Could you check a few things on this model? Use its own coordinates, in mm. A direction names the side the tool comes from. Round coordinates to 2 decimals unless told otherwise and drop trailing zeros. Order: outer loops, then holes, each group sorted by start corner. A loop starts at its lowest first (then second) coordinate and runs counter-clockwise, first axis right, second up. Notation, with made-up numbers: M -30.75,1 L 26.25,1 A17 ccw 26.25,17 Z; hole C 88.25,44.25 d3. An arc over 180 degrees is marked long. Write each question's results on one line, items separated by ' | '. Start each with the question number.
1. Suppose I cut it at A-A on y = 0. Write out the boundary of the cut face in (x, z), and give its area (3 significant figures).
2. Suppose I cut it at B-B on z = 4.5. Write out the boundary of the cut face in (x, y), and give its area (3 significant figures).
3. For faces 1 (the flat face through (1, 22.5, 4)), 2 (the cylindrical face through (21.1, -1.5, 2)), 3 (the cylindrical face through (9.89, 0.33, -1.05)), which set-ups out of +Z, -Z, +X, -X, +Y, -Y let a thin tool reach every point of the face, with its end or its side?
4. I'm going to push flat-ended pins straight in: pin 1 (2 mm diameter, centred on x = 20, z = 0, fed in from +Y); pin 2 (2 mm diameter, centred on x = 2.5, y = 19.5, fed in from +Z); pin 3 (0.8 mm diameter, centred on y = 0, z = 3.5, fed in from -X); pin 4 (2 mm diameter, centred on x = 22, y = 0, fed in from +Z). Where does each tip first touch, or does it pass through?
5. We'd pull the mould along Y, two halves only. Please class faces 4 (the flat face through (12, -27.5, 0)), 5 (the conical face through (19.72, 16.58, -0.04)), 6 (the flat face through (4.5, -19, 4)): released by +Y, released by -Y, zero draft, split by the parting line, or undercut.
6. Please list where these lines run through material, in increasing order: L1, parallel to X at y = 21.5, z = 0; L2, parallel to Y at x = 2, z = 0.25; L3, parallel to Y at x = 13, z = 0.
from build123d import *

# Parameters (mm, degrees)
SKETCH_1_W                  = 12
SKETCH_1_H                  = 55
EXTRUDE_1_DEPTH             = 25
SKETCH_2_R                  = 1.1
CUT_EXTRUDE_1_DEPTH         = 25
SKETCH_3_R                  = 2.5
CUT_EXTRUDE_2_DEPTH         = 8
SKETCH_4_W                  = 24
SKETCH_4_H                  = 3
CUT_EXTRUDE_3_DEPTH         = 6
HOLE_WIZARD_M4_1_AT_2_COUNT = 2
HOLE_WIZARD_M4_1_AT_2_PITCH = 15
FILLET_1_R                  = 1
CUT_EXTRUDE_4_DEPTH         = 4
HOLE_WIZARD_M3_1_D          = 2.5
FILLET_2_R                  = 1


with BuildPart() as part:
    # 草图1 → 凸台-拉伸1 (new body)
    with BuildSketch(Plane(origin=(0, 0, 0), x_dir=(0, 0, -1), z_dir=(1, 0, 0))):
        Rectangle(SKETCH_1_W, SKETCH_1_H)
    extrude(amount=EXTRUDE_1_DEPTH)

    # 草图2 → 切除-拉伸1 (cut)
    with BuildSketch(Plane(origin=(25, 0, 0), x_dir=(0, 0, -1), z_dir=(1, 0, 0))):
        Circle(SKETCH_2_R)
    extrude(amount=-CUT_EXTRUDE_1_DEPTH, mode=Mode.SUBTRACT)

    # 草图3 → 切除-拉伸2 (cut)
    with BuildSketch(Plane(origin=(25, 0, 0), x_dir=(0, 0, -1), z_dir=(1, 0, 0))):
        Circle(SKETCH_3_R)
    extrude(amount=-CUT_EXTRUDE_2_DEPTH, mode=Mode.SUBTRACT)

    # 草图4 → 切除-拉伸3 (cut)
    with BuildSketch(Plane.XY.offset(6)):
        Rectangle(SKETCH_4_W, SKETCH_4_H)
    extrude(amount=-CUT_EXTRUDE_3_DEPTH, mode=Mode.SUBTRACT)

    # 草图7 → M4 螺纹孔1 (revolve, cut)
    with BuildSketch(Plane(origin=(5, 27.5, 0), x_dir=(0, 0, 1), z_dir=(1, 0, 0))):
        Polygon((0, 0), (0, 11.091420021), (1.65, 10.1), (1.65, 0), align=None)
    hole_wizard_m4_1 = revolve(axis=Axis((5, 33.85, 0), (0, -1, 0)), mode=Mode.SUBTRACT)

    # M4 螺纹孔1 at 2: M4 螺纹孔1 ×2
    with Locations(*[(i * HOLE_WIZARD_M4_1_AT_2_PITCH, 0, 0) for i in range(1, HOLE_WIZARD_M4_1_AT_2_COUNT)]):
        add(hole_wizard_m4_1, mode=Mode.SUBTRACT)

    # 镜向1: M4 螺纹孔1 across plane
    add(hole_wizard_m4_1.mirror(Plane.ZX), mode=Mode.SUBTRACT)

    # 镜向1 copy 1 sketch → 镜向1 copy 1 (revolve, cut)
    with BuildSketch(Plane(origin=(20, -27.5, 0), x_dir=(0, 0, 1), z_dir=(1, 0, 0))):
        Polygon((0, 0), (0, -11.091420021), (1.65, -10.1), (1.65, 0), align=None)
    revolve(axis=Axis((20, -33.85, 0), (0, -1, 0)), mode=Mode.SUBTRACT)

    # 圆角1
    fillet_1_edges = [part.edges().sort_by_distance(p)[0] for p in [
        (12, -1.5, 3),
        (12, 1.5, 3),
    ]]
    fillet(fillet_1_edges, radius=FILLET_1_R)

    # 草图9 → 切除-拉伸4 (cut)
    with BuildSketch(Plane.XY.offset(6)):
        with BuildLine():
            Line((-4.5, 22.5), (2.5, 22.5))
            ThreePointArc((2.5, 22.5), (3.914213562, 21.914213562), (4.5, 20.5))
            Line((4.5, 20.5), (4.5, 17.5))
            ThreePointArc((4.5, 17.5), (3.914213562, 16.085786438), (2.5, 15.5))
            Line((2.5, 15.5), (-4.5, 15.5))
            Line((-4.5, 15.5), (-4.5, 22.5))
        make_face()
    cut_extrude_4 = extrude(amount=-CUT_EXTRUDE_4_DEPTH, mode=Mode.SUBTRACT)

    # 镜向2: 切除-拉伸4 across plane
    add(cut_extrude_4.mirror(Plane.ZX), mode=Mode.SUBTRACT)

    # M3 螺纹孔1 (through all)
    with Locations(Plane.XY.offset(6)):
        with Locations((22, 0)):
            Hole(HOLE_WIZARD_M3_1_D / 2)

    # 圆角2
    fillet_2_edges = [part.edges().sort_by_distance(p)[0] for p in [
        (17, 0, 1.1),
    ]]
    fillet(fillet_2_edges, radius=FILLET_2_R)


solid = part.part
Filled sheet:
1) outline: M 0,-6 L 20.75,-6 L 20.75,-2.5 L 17,-2.5 L 17,-2.1 A1 ccw 16,-1.1 L 0,-1.1 Z; M 12,1.1 L 16,1.1 A1 ccw 17,2.1 L 17,2.5 L 20.75,2.5 L 20.75,6 L 12,6 Z; M 23.25,-6 L 25,-6 L 25,-2.5 L 23.25,-2.5 Z; M 23.25,2.5 L 25,2.5 L 25,6 L 23.25,6 Z | area: 146 mm^2
2) outline: M 0,-27.5 L 25,-27.5 L 25,27.5 L 0,27.5 L 0,22.5 L 2.5,22.5 A2 cw 4.5,20.5 L 4.5,17.5 A2 cw 2.5,15.5 L 0,15.5 L 0,1.5 L 11,1.5 A1 cw 12,0.5 L 12,-0.5 A1 cw 11,-1.5 L 0,-1.5 L 0,-15.5 L 2.5,-15.5 A2 cw 4.5,-17.5 L 4.5,-20.5 A2 cw 2.5,-22.5 L 0,-22.5 Z; hole C 22,0 d2.5 | area: 1,270 mm^2
3) face 1: +Z, -X | face 2: +X | face 3: +X, -X
4) pin 1: stops at y = 17.01 | pin 2: stops at z = 2 | pin 3: stops at x = 12 | pin 4: passes through
5) face 4: released by -Y | face 5: released by +Y | face 6: undercut
6) L1: x = 0 to 3.35, 6.65 to 18.35, 21.65 to 25 | L2: y = -27.5 to -1.5, 1.5 to 27.5 | L3: y = -27.5 to -1.1, 1.1 to 27.5
